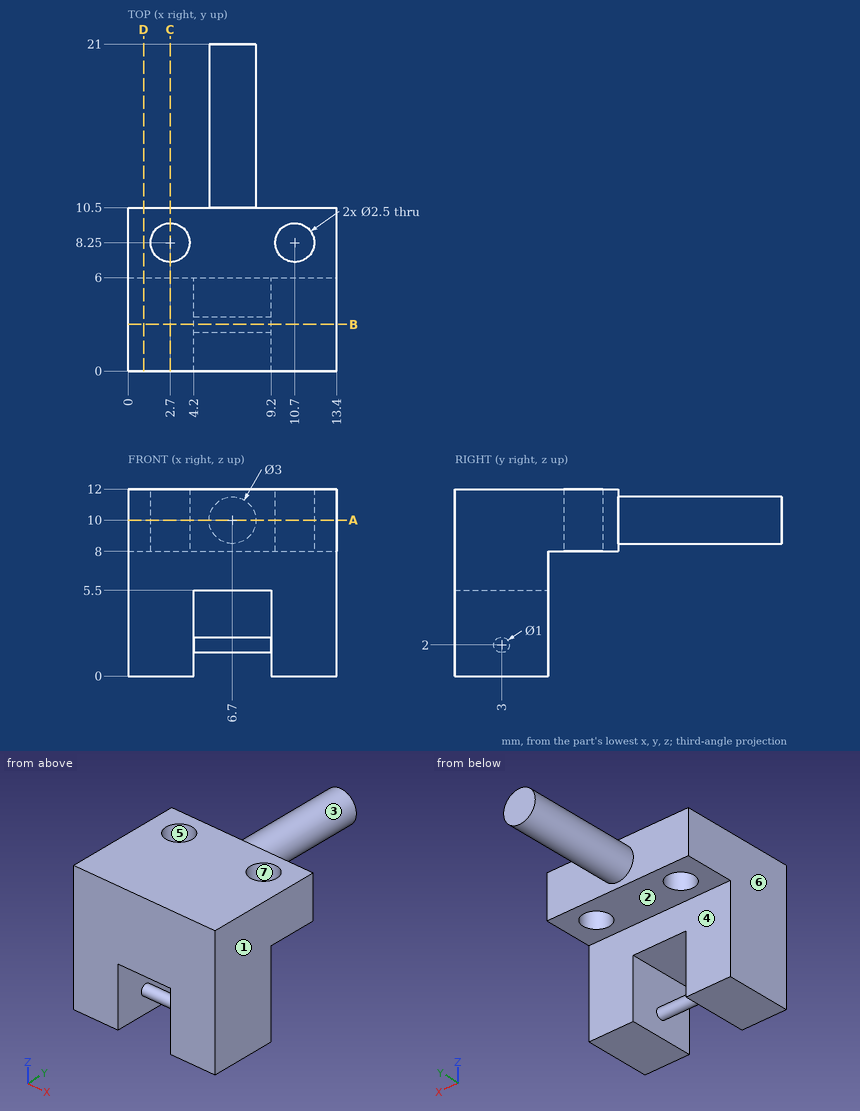
The figure shows three views and two pictorial views of one solid part (mm, origin at its lowest corner). Answer the questions. A direction names the side the tool comes from. Round coordinates to 2 decimals unless told otherwise and drop trailing zeros. Write each loop counter-clockwise with the first axis right and the second up, starting at its lowest first coordinate (ties: lowest second). Pieces come first, ordered by that corner, then holes. Notation, with made-up numbers: (26.5, 46.5) - (56.5, 46.5) arc R9 ccw to (56.5, 58.5) - close; hole circle Ø8 at (22, 18). An arc over 180 degrees is marked (long way). Use one line per item in the form item = value. Start each with the question number.
Item 1: Flat-ended cylindrical pins translate along their axes: pin 1 Ø2 at (x, y) = (2.7, 8.25) entering from +Z; pin 2 Ø1 at (x, y) = (7.5, 16) entering from +Z; pin 3 Ø2 at (x, y) = (7, 9.5) entering from -Z. Find the tip coordinate at first contact, or state that the pin passes through.
Item 2: Determine the mould class of the marked faces 4, 5, 6 and 7 for opening direction Y: +Y half, -Y half, draft (parallel to the pull), parting line (faces both ways), or undercut.
Item 3: A cutting plane is placed at B-B (y = 3). Write down the section's boundary in (x, z).
Item 4: A tool of negligible diameter and unlimited length cuts with its end or side. For the marked faces 1, 2 and 3, from which of +Z, -Z, +X, -X, +Y, -Y can it reach the whole face along a straight path? Write none if from no direction.
Item 5: A cutting plane is placed at D-D (x = 1). Write down the section's boundary in (y, z).
Item 6: Find the intervals of material crossed by line 1 (Y direction, x = 10.7, z = 9.3); line 2 (X direction, y = 2, z = 4.75); line 3 (Y direction, x = 1.75, z = 1), in increasing order. Write a range as [from, to].
Item 7: A cutting plane is placed at A-A (z = 10). Write down the section's boundary in (x, y), plus the area to 3 significant figures.
Item 8: A cutting plane is placed at C-C (x = 2.7). Write down the section's boundary in (y, z).
The answers:
q1.pin_1 = through
q1.pin_2 = 11.47
q1.pin_3 = 8
q2.face_4 = +Y half
q2.face_5 = undercut
q2.face_6 = draft
q2.face_7 = undercut
q3.outline = (0, 0) - (4.2, 0) - (4.2, 1.5) - (9.2, 1.5) - (9.2, 0) - (13.4, 0) - (13.4, 12) - (0, 12) - close; hole (4.2, 2.5) - (9.2, 2.5) - (9.2, 5.5) - (4.2, 5.5) - close
q4.face_1 = +Z, -Z, +X, +Y, -Y
q4.face_2 = -Z, +X, -X, +Y
q4.face_3 = +Y
q5.outline = (0, 0) - (6, 0) - (6, 8) - (10.5, 8) - (10.5, 12) - (0, 12) - close
q6.line_1 = [0, 7], [9.5, 10.5]
q6.line_2 = [0, 4.2], [9.2, 13.4]
q6.line_3 = [0, 6]
q7.outline = (0, 0) - (13.4, 0) - (13.4, 10.5) - (8.2, 10.5) - (8.2, 21) - (5.2, 21) - (5.2, 10.5) - (0, 10.5) - close; hole circle Ø2.5 at (2.7, 8.25); hole circle Ø2.5 at (10.7, 8.25)
q7.area = 162 mm^2
q8.outline = (0, 0) - (6, 0) - (6, 8) - (7, 8) - (7, 12) - (0, 12) - close; (9.5, 8) - (10.5, 8) - (10.5, 12) - (9.5, 12) - close
